Source: three-view drawing plus pictorial views. Frame: mm from the lowest corner of the part. A direction names the side the tool comes from. Give positions to 0.01 mm unless a question says otherwise; leave off trailing zeros. Order: outer loops, then holes, each group sorted by start corner. A loop starts at its lowest first (then second) coordinate and runs counter-clockwise, first axis right, second up. Notation, with made-up numbers: (28, 70.5) -> (46, 70.5) arc R27 cw to (46, 94.5) -> close; hole circle Ø11 at (33.25, 56). An arc over 180 degrees is marked (long way). Write item = value, one per line.
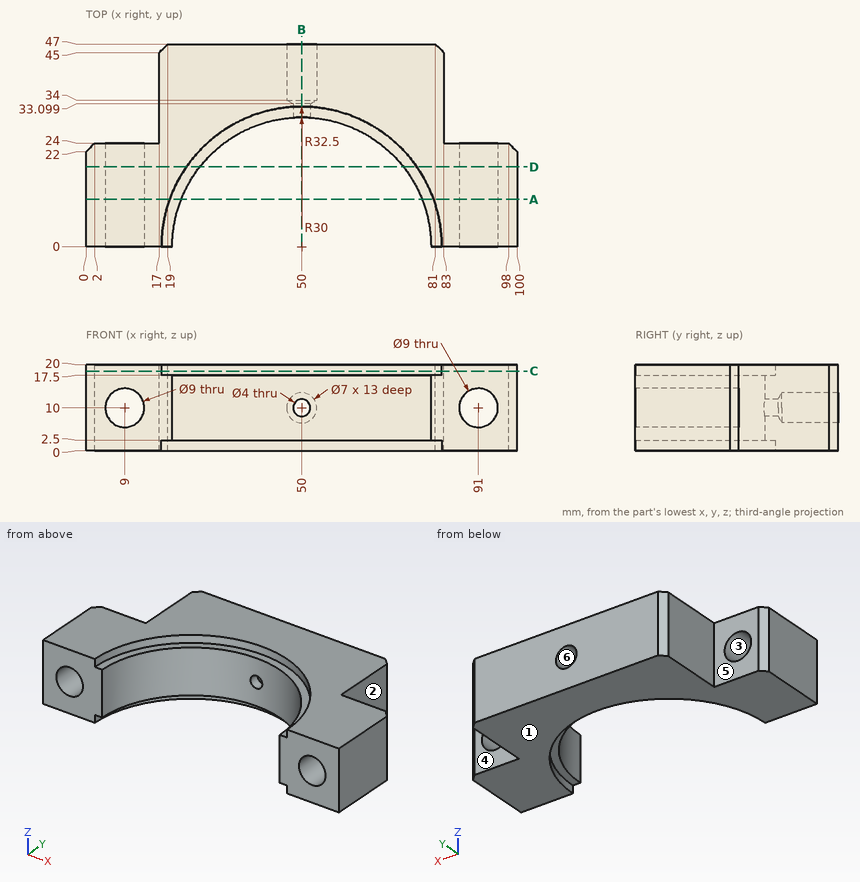
1) Section query A-A (y = 11). Output: boundary loops of the cut face in (x, z).
Check sheet entries:
outline = (0, 0) -> (19.42, 0) -> (19.42, 2.5) -> (22.09, 2.5) -> (22.09, 17.5) -> (19.42, 17.5) -> (19.42, 20) -> (0, 20) -> close; (77.91, 2.5) -> (80.58, 2.5) -> (80.58, 0) -> (100, 0) -> (100, 20) -> (80.58, 20) -> (80.58, 17.5) -> (77.91, 17.5) -> close; hole circle Ø9 at (9, 10); hole circle Ø9 at (91, 10)
2) Reachability of the marked faces 4, 5 and 6 from +Z, -Z, +X, -X, +Y, -Y: full face, straight path, thin tool, end or side. Return the list, or none.
Check sheet entries:
face_4 = +Z, -Z, +X, +Y
face_5 = +Z, -Z, -X, +Y
face_6 = +Y
3) Line query: line 1 (Z direction, x = 9, y = 8); line 2 (X direction, y = 32, z = 10); line 3 (Z direction, x = 50, y = 32.1). Output: solid intervals per line, ascending. Write a range as from..to.
Check sheet entries:
line_1 = 0..5.5, 14.5..20
line_2 = 17..48, 52..83
line_3 = 2.5..8, 12..17.5
4) Section query D-D (y = 18.5). Output: boundary loops of the cut face in (x, z), plus the area to 3 significant figures.
Check sheet entries:
outline = (0, 0) -> (23.28, 0) -> (23.28, 2.5) -> (26.38, 2.5) -> (26.38, 17.5) -> (23.28, 17.5) -> (23.28, 20) -> (0, 20) -> close; (73.62, 2.5) -> (76.72, 2.5) -> (76.72, 0) -> (100, 0) -> (100, 20) -> (76.72, 20) -> (76.72, 17.5) -> (73.62, 17.5) -> close; hole circle Ø9 at (9, 10); hole circle Ø9 at (91, 10)
area = 897 mm²
5) Section query B-B (x = 50). Output: boundary loops of the cut face in (y, z).
Check sheet entries:
outline = (30, 2.5) -> (32.5, 2.5) -> (32.5, 0) -> (47, 0) -> (47, 6.5) -> (34, 6.5) -> (33.1, 8) -> (30, 8) -> close; (30, 12) -> (33.1, 12) -> (34, 13.5) -> (47, 13.5) -> (47, 20) -> (32.5, 20) -> (32.5, 17.5) -> (30, 17.5) -> close
6) Section query C-C (z = 18.5). Output: boundary loops of the cut face in (x, y), plus the area to 3 significant figures.
Check sheet entries:
outline = (0, 0) -> (17.5, 0) arc R32.5 cw to (82.5, 0) -> (100, 0) -> (100, 22) -> (98, 24) -> (83, 24) -> (83, 45) -> (81, 47) -> (19, 47) -> (17, 45) -> (17, 24) -> (2, 24) -> (0, 22) -> close
area = 2,250 mm²
7) Mould query, pull axis X, two halves, no side actions, for the marked faces 1, 2 and 3. Classes: +X half, -X half, draft (parallel to the pull), parting line (faces both ways), or undercut.
Check sheet entries:
face_1 = draft
face_2 = +X half
face_3 = undercut
8) First-contact query: P1, Ø2, axis at x = 14.5, y = 30, coming from the -Z side; P2, Ø2, axis at y = 36.5, z = 10, coming from the -X side; P3, Ø9, axis at x = 50, z = 10, coming from the -Y side; P4, Ø1, axis at x = 45.5, z = 5, coming from the -Y side. Flat tips, straight axial feed; report the tip coordinate or a pass-through.
Check sheet entries:
P1 = through
P2 = 17
P3 = 29.66
P4 = 29.58
